Geometry: final body of the model. Coordinates: model frame, mm. A direction names the side the tool comes from. Round coordinates to 2 decimals unless told otherwise and drop trailing zeros. Loops run counter-clockwise (first coordinate to the right, second up) from the corner with the lowest first, then second, coordinate; pieces in that order, holes last. Notation, with made-up numbers: (13.5, 73.5) -> (60.5, 73.5) arc R18 ccw to (60.5, 106.5) -> close; hole circle Ø7 at (54, 77.25). An arc over 180 degrees is marked (long way). Answer in a Markdown table with one row per item.
```python
from build123d import *

# Parameters (mm, degrees)
SKETCH_1_W               = 1457
SKETCH_1_H               = 472
EXTRUDE_1_DEPTH          = 30
SHELL_1_T                = -2
SKETCH_2_W               = 1457
SKETCH_2_H               = 492
SKETCH_2_W_2             = 1417
SKETCH_2_H_2             = 450
EXTRUDE_2_DEPTH          = 2
CUT_EXTRUDE_1_DEPTH      = 1501
CUT_EXTRUDE_1_DEPTH_BACK = 10
SKETCH_3_R               = 4.5
SKETCH_6_R               = 4.5
CUT_EXTRUDE_2_DEPTH      = 10


with BuildPart() as part:
    # 草图1 → 凸台-拉伸1 (new body)
    with BuildSketch(Plane.XY):
        with Locations((728.5, 236)):
            Rectangle(SKETCH_1_W, SKETCH_1_H)
    extrude(amount=EXTRUDE_1_DEPTH)

    # 抽壳1
    shell_1_openings = [part.faces().sort_by_distance(p)[0] for p in [
        (728.5, 236, 30),
    ]]
    offset(amount=SHELL_1_T, openings=shell_1_openings, kind=Kind.INTERSECTION)

    # 草图2 → 凸台-拉伸2 (add)
    with BuildSketch(Plane.XY.offset(30)):
        with Locations((728.5, 246)):
            Rectangle(SKETCH_2_W, SKETCH_2_H)
        with Locations((728.5, 245)):
            Rectangle(SKETCH_2_W_2, SKETCH_2_H_2, mode=Mode.SUBTRACT)
    extrude(amount=-EXTRUDE_2_DEPTH)

    # 草图3 → 切除-拉伸1 (cut, two sides: drawn at the far end of the back side and taken through both)
    with BuildSketch(Plane(origin=(2, 0, 0), x_dir=(0, 0, -1), z_dir=(1, 0, 0)).offset(-CUT_EXTRUDE_1_DEPTH_BACK)):
        with Locations(Location((-16, 442, 0), (0, 0, 180))):
            Circle(SKETCH_3_R)
        with Locations(Location((-16, 30, 0), (0, 0, 180))):
            Circle(SKETCH_3_R)
    extrude(amount=CUT_EXTRUDE_1_DEPTH + CUT_EXTRUDE_1_DEPTH_BACK, mode=Mode.SUBTRACT)

    # 草图6 → 切除-拉伸2 (cut)
    with BuildSketch(Plane(origin=(0, 2, 0), x_dir=(1, 0, 0), z_dir=(0, 1, 0))):
        with Locations(Location((30, -16, 0), (0, 0, 270))):
            Circle(SKETCH_6_R)
        with Locations(Location((450, -16, 0), (0, 0, 270))):
            Circle(SKETCH_6_R)
        with Locations(Location((1427, -16, 0), (0, 0, 270))):
            Circle(SKETCH_6_R)
        with Locations(Location((968.5, -16, 0), (0, 0, 270))):
            Circle(SKETCH_6_R)
        with Locations(Location((510, -16, 0), (0, 0, 270))):
            Circle(SKETCH_6_R)
        with Locations(Location((78, -16, 0), (0, 0, 270))):
            Circle(SKETCH_6_R)
        with Locations(Location((178, -16, 0), (0, 0, 270))):
            Circle(SKETCH_6_R)
    extrude(amount=-CUT_EXTRUDE_2_DEPTH, mode=Mode.SUBTRACT)


solid = part.part
```
Item 1: Set-up query: faces 4 (the flat face through (2, 233, 15)), 5 (the flat face through (725, 484, 30)), 6 (the flat face through (718, 472, 14)). Return all of +Z, -Z, +X, -X, +Y, -Y with unobstructed straight access to the full face (end or side cutting, diameter ignored); none if empty.
Ans:
| item | result |
|---|---|
| face 4 | none |
| face 5 | +Z, +X, -X, +Y, -Y |
| face 6 | -Z, +X, -X, +Y |
Item 2: Section query B-B, the plane x = 356. Output: boundary loops of the cut face in (y, z), and give its area (3 significant figures).
Ans:
| item | result |
|---|---|
| outline | (0, 0) -> (472, 0) -> (472, 28) -> (492, 28) -> (492, 30) -> (470, 30) -> (470, 2) -> (2, 2) -> (2, 28) -> (20, 28) -> (20, 30) -> (0, 30) -> close |
| area | 1,130 mm2 |
Item 3: Mould query, pull axis Y, two halves, no side actions, for faces 1 (the flat face through (1457, 243, 15)), 2 (the flat face through (725, 12, 28)), 3 (the flat face through (718, 0, 15)). Classes: released by +Y, released by -Y, zero draft, split by the parting line, or undercut.
Ans:
| item | result |
|---|---|
| face 1 | zero draft |
| face 2 | undercut |
| face 3 | released by -Y |
Item 4: Ray query, L1, parallel to Y at x = 539, z = 20.75; L2, parallel to X at y = 337, z = 13.5; L3, parallel to Y at x = 1456.65, z = 16. Return the intervals inside material, ascending.
Ans:
| item | result |
|---|---|
| L1 | 0 to 2, 470 to 472 |
| L2 | 0 to 2, 1455 to 1457 |
| L3 | 0 to 25.5, 34.5 to 437.5, 446.5 to 472 |
Item 5: Section query C-C, the plane y = 102. Output: boundary loops of the cut face in (x, z).
Ans:
| item | result |
|---|---|
| outline | (0, 0) -> (1457, 0) -> (1457, 30) -> (1437, 30) -> (1437, 28) -> (1455, 28) -> (1455, 2) -> (2, 2) -> (2, 28) -> (20, 28) -> (20, 30) -> (0, 30) -> close |
Item 6: First-contact query: P1, Ø5.5, axis at x = 178, z = 16, coming from the -Y side; P2, Ø3, axis at y = 253, z = 10, coming from the -X side; P3, Ø5.5, axis at x = 1427, z = 16, coming from the +Y side; P4, Ø12, axis at x = 1139.5, y = 57.5, coming from the +Z side. Flat tips, straight axial feed; report the tip coordinate or a pass-through.
Ans:
| item | result |
|---|---|
| P1 | y = 470 |
| P2 | x = 0 |
| P3 | y = 472 |
| P4 | z = 2 |
Item 7: Section query A-A, the plane z = 7. Output: boundary loops of the cut face in (x, y), and give its area (3 significant figures).
Ans:
| item | result |
|---|---|
| outline | (0, 0) -> (1457, 0) -> (1457, 472) -> (0, 472) -> close; hole (2, 2) -> (1455, 2) -> (1455, 470) -> (2, 470) -> close |
| area | 7,700 mm2 |
